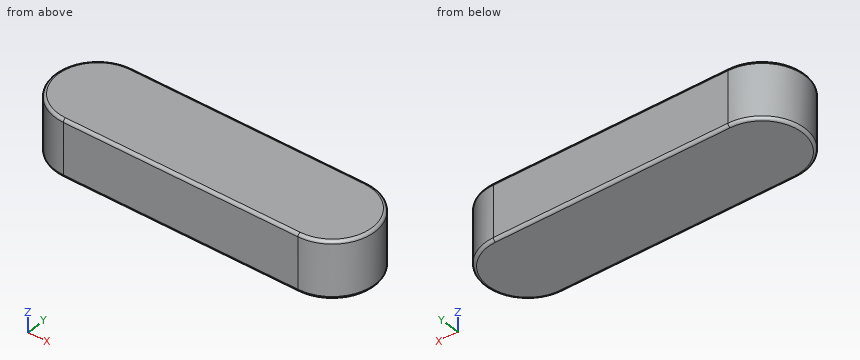
from build123d import *

# Parameters (mm, degrees)
BOSS_EXTRUDE_DEPTH = 8
FILLET1_R          = 0.4


with BuildPart() as part:
    # Sketch1 → Boss-Extrude (new body)
    with BuildSketch(Plane.XY):
        with BuildLine():
            Line((-16.5, 6), (16.5, 6))
            ThreePointArc((16.5, 6), (22.5, 0), (16.5, -6))
            Line((16.5, -6), (-16.5, -6))
            ThreePointArc((-16.5, -6), (-22.5, 0), (-16.5, 6))
        make_face()
    extrude(amount=BOSS_EXTRUDE_DEPTH)

    # Fillet1
    fillet1_edges = [part.edges().sort_by_distance(p)[0] for p in [
        (22.5, 0, 8),
        (0, 6, 8),
        (-22.5, 0, 8),
        (0, 6, 0),
        (22.5, 0, 0),
        (0, -6, 0),
        (-22.5, 0, 0),
        (0, -6, 8),
    ]]
    fillet(fillet1_edges, radius=FILLET1_R)


solid = part.part
Here's how the part is built. I have some questions about the finished solid (model axes, mm). Give positions to 0.01 mm unless a question says otherwise; leave off trailing zeros. Order: outer loops, then holes, each group sorted by start corner. A loop starts at its lowest first (then second) coordinate and runs counter-clockwise, first axis right, second up. Notation, with made-up numbers: M -29,68 L 13,68 A26 cw 13,100 Z; hole C -25,-16 d7. An arc over 180 degrees is marked long. Answer as a JSON object with one key per item and string values. Group by question number.
1) Suppose I cut it at A-A, the plane z = 4.25. Write out the boundary of the cut face in (x, y), plus the area to 3 significant figures.
2) Please list where these lines run through material, in increasing order: L1, parallel to X at y = 4, z = 3.75; L2, parallel to X at y = -1.5, z = 3.75; L3, parallel to Y at x = -18, z = 4.5. Write a range as [from, to].
3) I'm going to push a flat-ended pin straight in: pin 1 Ø3 at (y, z) = (4.5, 5) entering from +X. Where does the tip first touch, or does it pass through?
Results found:
{
 "1": {"outline": "M -16.5,-6 L 16.5,-6 A6 ccw 16.5,6 L -16.5,6 A6 ccw Z", "area": "509 mm²"},
 "2": {"L1": "[-20.97, 20.97]", "L2": "[-22.31, 22.31]", "L3": "[-5.81, 5.81]"},
 "3": {"pin 1": "x = 21.7"}
}
